```python
from build123d import *

# Parameters (mm, degrees)
CENTRE_CUT_SKETCH_R = 6
CENTRE_CUT_DEPTH    = 108.301863917


with BuildPart() as part:
    # Disc Profile Sketch → Stepped Disc Revolve (revolve)
    with BuildSketch(Plane.XY, mode=Mode.PRIVATE) as stepped_disc_revolve_sk:
        with BuildLine():
            Line((0, 0), (0, 30))
            Line((0, 30), (2, 30))
            Line((2, 30), (2, 45))
            Line((2, 45), (22, 45))
            Line((22, 45), (22, 32))
            ThreePointArc((22, 32), (22.585786438, 30.585786438), (24, 30))
            Line((24, 30), (59, 30))
            Line((59, 30), (59, 23.7))
            Line((59, 23.7), (74, 23.7))
            Line((74, 23.7), (74, 0))
            Line((74, 0), (0, 0))
        make_face()
    revolve(stepped_disc_revolve_sk.sketch.rotate(Axis((0, 0, 0), (0, 1, 0)), 90), axis=Axis((0, 0, 0), (0, 1, 0)))

    # Centre Cut Sketch → Centre Cut (cut, through all)
    with BuildSketch(Plane(origin=(0, 23.7, 0), x_dir=(1, 0, 0), z_dir=(0, 1, 0))):
        with Locations(Location((-45, 0, 0), (0, 0, 270))):
            Circle(CENTRE_CUT_SKETCH_R)
        with Locations(Location((45, 0, 0), (0, 0, 270))):
            Circle(CENTRE_CUT_SKETCH_R)
    extrude(amount=-CENTRE_CUT_DEPTH, mode=Mode.SUBTRACT)


solid = part.part
```
Design review of the part built by this model. Coordinates are the model's own, in mm. A direction names the side the tool comes from. Give positions to 0.01 mm unless a question says otherwise; leave off trailing zeros. Order: outer loops, then holes, each group sorted by start corner. A loop starts at its lowest first (then second) coordinate and runs counter-clockwise, first axis right, second up. Notation, with made-up numbers: M 63.25,48 L 105.25,48 A14 cw 105.25,67 Z; hole C 15.25,-23.75 d1. An arc over 180 degrees is marked long. One line per question, with ' | ' between items. Start each with the question number.
Q1. For pin 1 Ø10 at (y, z) = (13, 30.5) entering from -X; pin 2 Ø5 at (y, z) = (28, -16) entering from +X; pin 3 Ø10 at (y, z) = (32.5, -19.5) entering from +X; pin 4 Ø8 at (y, z) = (35.5, -58.5) entering from -X, all flat-tipped, find the tip position at first contact; note any pin that passes through.
Q2. Machinability: for faces 4 (the face through (-45, 23.7, 0)), 5 (the face through (33, 23.7, -50)), 6 (the face through (65.65, 11.68, -34.15)), which of the approach directions +Z, -Z, +X, -X, +Y, -Y give a long, thin tool a straight path to every point of the face, cutting with its end or side? Answer none if there is none.
Q3. We need section A-A (z = 0). Write out the cut boundary in (x, y).
Q4. We need section B-B (x = 0). Write out the cut boundary in (y, z), plus the area to 3 significant figures.
Q5. We need section D-D (y = 37). Write out the cut boundary in (x, z), plus the area to 3 significant figures.
Q6. We need section C-C (y = 8). Write out the cut boundary in (x, z), plus the area to 3 significant figures.
Q7. The part is to be moulded in two halves that separate along Z. For faces 1 (the face through (-50.857, 12.016, -1.301)), 2 (the face through (21.477, 38.409, 4.769)), 3 (the face through (-1, 0, 1)), say which applies: +Z half, -Z half, draft (parallel to the pull), parting line (faces both ways), or undercut.
Q8. For L1, parallel to X at y = 7.25, z = 0; L2, parallel to X at y = 38.25, z = 0; L3, parallel to Y at x = 58, z = 14, list the stretches that pass through material, from the lowest coordinate up. Write a range as [from, to].
Returned:
1) pin 1: x = -69.47 | pin 2: x = 57.43 | pin 3: x = 57.02 | pin 4: through
2) face 4: -Y | face 5: +Y | face 6: +Y, -Y
3) outline: M -74,0 L -51,0 L -51,23.7 L -39,23.7 L -39,0 L 39,0 L 39,23.7 L 51,23.7 L 51,0 L 74,0 L 74,23.7 L 59,23.7 L 59,30 L 24,30 A2 cw 22,32 L 22,45 L 2,45 L 2,30 L -2,30 L -2,45 L -22,45 L -22,32 A2 cw -24,30 L -59,30 L -59,23.7 L -74,23.7 Z
4) outline: M 0,-74 L 23.7,-74 L 23.7,-59 L 30,-59 L 30,-24 A2 cw 32,-22 L 45,-22 L 45,-2 L 30,-2 L 30,2 L 45,2 L 45,22 L 32,22 A2 cw 30,24 L 30,59 L 23.7,59 L 23.7,74 L 0,74 Z | area: 4,850 mm2
5) outline: C 0,0 d44; hole C 0,0 d4 | area: 1,510 mm2
6) outline: C 0,0 d148; hole C -45,0 d12; hole C 45,0 d12 | area: 17,000 mm2
7) face 1: undercut | face 2: parting line | face 3: draft
8) L1: [-74, -51], [-39, 39], [51, 74] | L2: [-22, -2], [2, 22] | L3: [0, 23.7]
